from build123d import *

# Parameters (mm, degrees)
SKETCH1_W             = 9
SKETCH1_H             = 35
BOSS_EXTRUDE1_DEPTH   = 21
M6_TAPPED_HOLE1_D     = 5
M6_TAPPED_HOLE1_DEPTH = 15
M6_TAPPED_HOLE1_TIP   = 1.502151548
M4_TAPPED_HOLE1_D     = 3.3
M4_TAPPED_HOLE1_DEPTH = 15
M4_TAPPED_HOLE1_TIP   = 0.991420021
FILLET1_R             = 1
CHAMFER1_SIZE         = 0.5


with BuildPart() as part:
    # Sketch1 → Boss-Extrude1 (new body)
    with BuildSketch(Plane.XY):
        with Locations((4.5, 0)):
            Rectangle(SKETCH1_W, SKETCH1_H)
    extrude(amount=BOSS_EXTRUDE1_DEPTH)

    # M6 Tapped Hole1
    with Locations(Plane(origin=(9, 0, 0), x_dir=(0, 0, -1), z_dir=(1, 0, 0))):
        with Locations((-10, 12.5), (-10, -12.5)):
            Hole(M6_TAPPED_HOLE1_D / 2, depth=M6_TAPPED_HOLE1_DEPTH)
            with Locations((0, 0, -(M6_TAPPED_HOLE1_DEPTH + M6_TAPPED_HOLE1_TIP / 2))):  # 118° drill point
                Cone(0, M6_TAPPED_HOLE1_D / 2, M6_TAPPED_HOLE1_TIP, mode=Mode.SUBTRACT)

    # M4 Tapped Hole1
    with Locations(Plane(origin=(0, 0, 0), x_dir=(-1, 0, 0), z_dir=(0, 0, -1))):
        with Locations((-4.5, 4.5), (-4.5, -4.5)):
            Hole(M4_TAPPED_HOLE1_D / 2, depth=M4_TAPPED_HOLE1_DEPTH)
            with Locations((0, 0, -(M4_TAPPED_HOLE1_DEPTH + M4_TAPPED_HOLE1_TIP / 2))):  # 118° drill point
                Cone(0, M4_TAPPED_HOLE1_D / 2, M4_TAPPED_HOLE1_TIP, mode=Mode.SUBTRACT)

    # Fillet1
    fillet1_edges = [part.edges().sort_by_distance(p)[0] for p in [
        (9, 0, 21),
        (0, 0, 21),
    ]]
    fillet(fillet1_edges, radius=FILLET1_R)

    # Chamfer1
    chamfer1_edges = [part.edges().sort_by_distance(p)[0] for p in [
        (9, 0, 0),
        (0, 0, 0),
    ]]
    chamfer(chamfer1_edges, length=CHAMFER1_SIZE)


solid = part.part
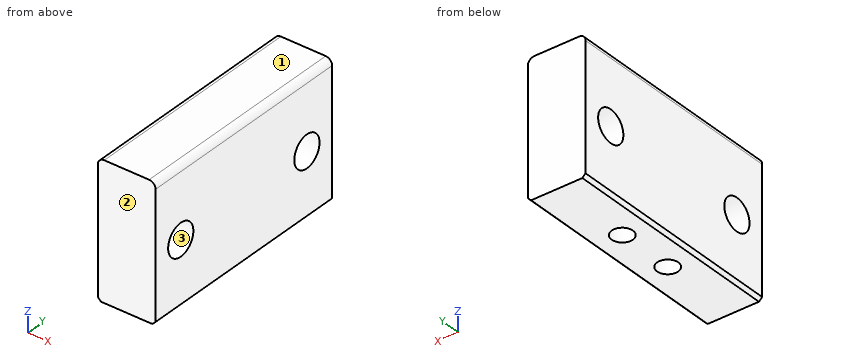
Geometry check sheet. Reference: the model listing, model coordinates, mm. Face numbers are marked on the shaded views. Coordinates: 2 decimals unless noted, no trailing zeros. Order: outer loops, then holes, each group sorted by start corner. A loop starts at its lowest first (then second) coordinate and runs counter-clockwise, first axis right, second up. Notation, with made-up numbers: (10, 12.5) - (16, 12.5) arc R26 ccw to (16, 40.5) - close; hole circle Ø8 at (39.25, -20.75). An arc over 180 degrees is marked (long way). One line per item, written item: value.
(1) Sectioned sample at C-C (x = 2.25). Enter the section's corners in (y, z).
Data:
outline: (-17.5, 0) - (17.5, 0) - (17.5, 21) - (-17.5, 21) - close; hole circle Ø5 at (-12.5, 10); hole circle Ø5 at (12.5, 10)
(2) Release check for a two-part mould opening along Z. For the marked faces 1, 2 and 3 record: +Z half, -Z half, draft (parallel to the pull), parting line (faces both ways), or undercut.
Data:
face 1: +Z half
face 2: draft
face 3: undercut
(3) Sectioned sample at D-D (z = 3.75). Enter the section's corners in (x, y), and give its area (3 significant figures).
Data:
outline: (0, -17.5) - (9, -17.5) - (9, 17.5) - (0, 17.5) - close; hole circle Ø3.3 at (4.5, -4.5); hole circle Ø3.3 at (4.5, 4.5)
area: 298 mm^2
(4) Thickness scan on probe 1 along Y at (x, z) = (4.5, 6.75); probe 2 along Y at (x, z) = (2.5, 10); probe 3 along Y at (x, z) = (4.5, 10). Record the ranges inside material, lowest first. Write a range as from..to.
Data:
probe 1: y = -17.5..-6.15, -2.85..2.85, 6.15..17.5
probe 2: y = -17.5..-15, -10..10, 15..17.5
probe 3: y = -17.5..-15, -10..-6.15, -2.85..2.85, 6.15..10, 15..17.5
(5) Depth check by flat-ended pin: pin 1 Ø3 at (x, y) = (4.5, 4.5) entering from -Z; pin 2 Ø2.5 at (x, y) = (4.5, -4.5) entering from -Z. Enter the tip coordinate at first touch or a pass-through.
Data:
pin 1: stops at z = 15.09
pin 2: stops at z = 15.24
(6) Sectioned sample at B-B (y = 12.5). Enter the section's corners in (x, z), and give its area (3 significant figures).
Data:
outline: (0, 0.5) - (0.5, 0) - (8.5, 0) - (9, 0.5) - (9, 7.5) - (0, 7.5) - close; (0, 12.5) - (9, 12.5) - (9, 20) arc R1 ccw to (8, 21) - (1, 21) arc R1 ccw to (0, 20) - close
area: 143 mm^2
(7) Sectioned sample at A-A (z = 10). Enter the section's corners in (x, y).
Data:
outline: (0, -17.5) - (9, -17.5) - (9, -15) - (0, -15) - close; (0, -10) - (9, -10) - (9, 10) - (0, 10) - close; (0, 15) - (9, 15) - (9, 17.5) - (0, 17.5) - close; hole circle Ø3.3 at (4.5, -4.5); hole circle Ø3.3 at (4.5, 4.5)
